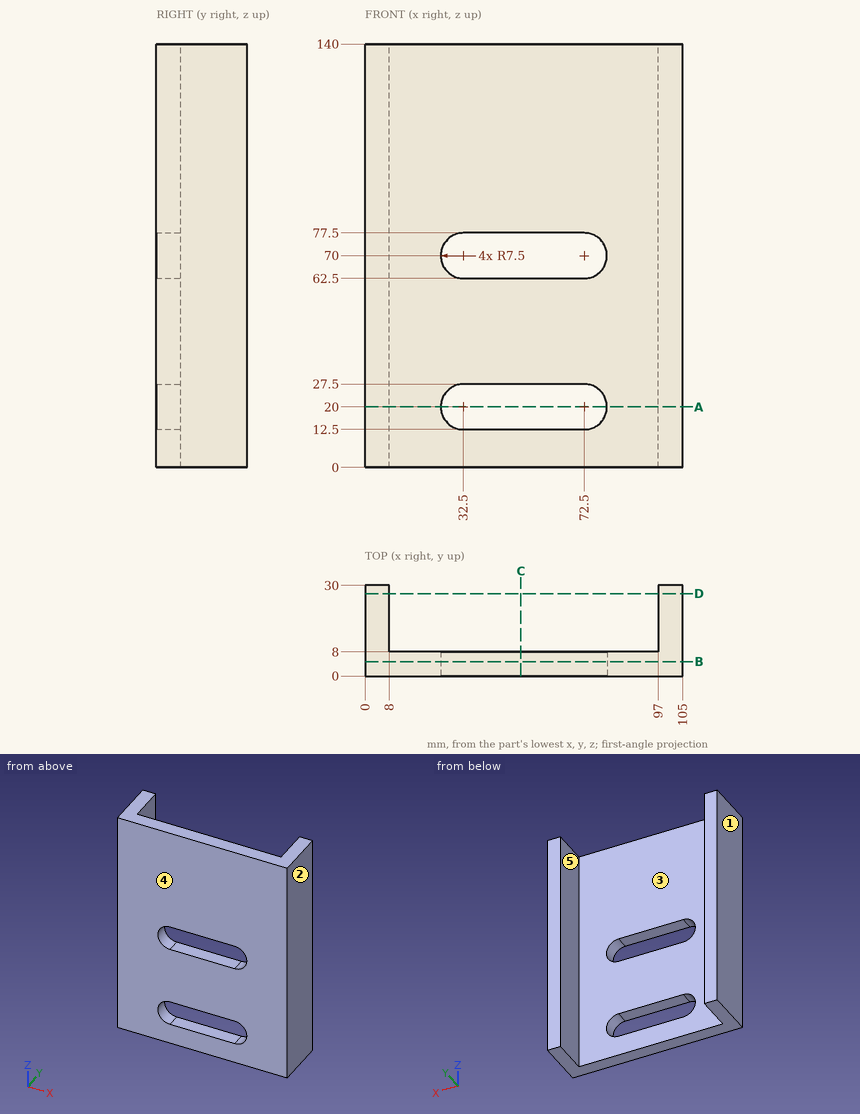
Part print with two shaded views. Sizes in mm from the minimum x, y, z corner. A direction names the side the tool comes from. Round coordinates to 2 decimals unless told otherwise and drop trailing zeros. Order: outer loops, then holes, each group sorted by start corner. A loop starts at its lowest first (then second) coordinate and runs counter-clockwise, first axis right, second up. Notation, with made-up numbers: (13, -13.75) - (72, -13.75) arc R25 cw to (72, 4.25) - close; hole circle Ø2 at (66, 61.25). An arc over 180 degrees is marked (long way). Answer as CSV lines item,"result". Start each with the question number.
1. Saw through at D-D, the plane y = 27.25. Write the cut outline in (x, z), and give its area (3 significant figures).
2. Pull direction X, two halves, no side cores. Call the marked faces 1, 2 and 3: +X half, -X half, draft (parallel to the pull), parting line (faces both ways), or undercut.
3. Saw through at B-B, the plane y = 4.75. Write the cut outline in (x, z).
4. Drill centre lines: L1, parallel to Z at x = 40.5, y = 4.5; L2, parallel to X at y = 13.5, z = 65; L3, parallel to Z at x = 75, y = 3.5. Where is each one in solid material? Low to high. Write a range as [from, to].
5. Saw through at C-C, the plane x = 51.5. Write the cut outline in (y, z), and give its area (3 significant figures).
6. Saw through at A-A, the plane z = 20. Write the cut outline in (x, y), and give its area (3 significant figures).
7. Pin check, flat tip, straight feed: pin 1 (8 mm diameter, centred on x = 31.5, z = 61.5, fed in from +Y). Stop position of the tip, or through.
8. Tool access for the marked faces 4 and 5: list every direction of +Z, -Z, +X, -X, +Y, -Y with a clear straight run to the whole face (end or side of a thin tool).
Model answer:
1,outline,"(0, 0) - (8, 0) - (8, 140) - (0, 140) - close; (97, 0) - (105, 0) - (105, 140) - (97, 140) - close"
1,area,"2,240 mm²"
2,face 1,"-X half"
2,face 2,"+X half"
2,face 3,"undercut"
3,outline,"(0, 0) - (105, 0) - (105, 140) - (0, 140) - close; hole (32.5, 12.5) - (72.5, 12.5) arc R7.5 ccw to (72.5, 27.5) - (32.5, 27.5) arc R7.5 ccw to start; hole (32.5, 62.5) - (72.5, 62.5) arc R7.5 ccw to (72.5, 77.5) - (32.5, 77.5) arc R7.5 ccw to start"
4,L1,"z = [0, 12.5], [27.5, 62.5], [77.5, 140]"
4,L2,"x = [0, 8], [97, 105]"
4,L3,"z = [0, 12.93], [27.07, 62.93], [77.07, 140]"
5,outline,"(0, 0) - (8, 0) - (8, 12.5) - (0, 12.5) - close; (0, 27.5) - (8, 27.5) - (8, 62.5) - (0, 62.5) - close; (0, 77.5) - (8, 77.5) - (8, 140) - (0, 140) - close"
5,area,"880 mm²"
6,outline,"(0, 0) - (25, 0) - (25, 8) - (8, 8) - (8, 30) - (0, 30) - close; (80, 0) - (105, 0) - (105, 30) - (97, 30) - (97, 8) - (80, 8) - close"
6,area,"752 mm²"
7,pin 1,"stops at y = 8"
8,face 4,"+Z, -Z, +X, -X, -Y"
8,face 5,"+Z, -Z, +Y"
